For this review, take the finished solid that the model builds, in its own axes (mm). Face numbers are marked on the shaded views. A direction names the side the tool comes from. Round coordinates to 2 decimals unless told otherwise and drop trailing zeros. Loops run counter-clockwise (first coordinate to the right, second up) from the corner with the lowest first, then second, coordinate; pieces in that order, holes last.
1) Tool access review of the marked faces 1, 2 and 3: name each direction out of +Z, -Z, +X, -X, +Y, -Y from which nothing blocks a thin tool from reaching the whole face with its end or side.
2) Take a section at A-A (y = 15.5). State the section outline as (x, z) points, then the cut area to 3 significant figures.
3) Take a section at D-D (y = 35). State the section outline as (x, z) points, then the cut area to 3 significant figures.
4) Take a section at B-B (x = 62). State the section outline as (y, z) points, then the cut area to 3 significant figures.
5) Wall thickness on L1, parallel to X at y = 29.5, z = 12.5; L2, parallel to Y at x = -72, z = -15; L3, parallel to X at y = 12, z = 18: over which ranges is each line inside the solid? List them lowest first.
6) Mouldability with a two-part tool opening along X and no side actions: class the marked faces 4, 5 and 6 as pulls with the +X half, pulls with the -X half, needs draft (parallel to the pull), parting line crosses it, or undercut.
7) Insertion check: pin 1 (7 mm diameter, centred on y = 27, z = 1, fed in from +X); pin 2 (2 mm diameter, centred on y = 62, z = 10, fed in from +X); pin 3 (4 mm diameter, centred on x = -6.5, z = -5, fed in from +Y); pin 4 (8 mm diameter, centred on x = 14, y = 69.5, fed in from -Z). Each pin has a flat end and moves straight along its axis. Give the tip position at first contact, or say it passes through.
8) Take a section at C-C (z = -9). State the section outline as (x, y) points, then the cut area to 3 significant figures.
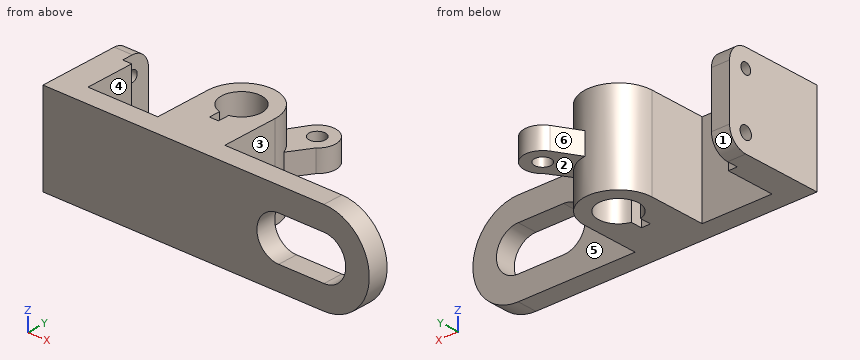
```python
from build123d import *

# Parameters (mm, degrees)
BASE_PLATE_11MM_DEPTH    = 11
UPRIGHT_BLOCK_DEPTH      = 50
CHANNEL_CUT_DEPTH        = 50
FRONT_WALL_12MM_DEPTH    = 6
WALL_HOLE_SKETCH_R       = 4.5
WALL_THROUGH_HOLE_DEPTH  = 69
BORE_KEYWAY_CUT_DEPTH    = 69
HOUSING_PAD_SKETCH_W     = 15
HOUSING_PAD_SKETCH_H     = 50
HOUSING_PAD_DEPTH        = 27
BORE_HOUSING_SKETCH_W    = 10
BORE_HOUSING_SKETCH_H    = 16
BORE_HOUSING_DEPTH       = 50
HOUSING_FILLET_R10_A_R   = 10
HOUSING_FILLET_R10_B_R   = 10
CROSS_HOLE_SKETCH_R      = 3.5
CROSS_HOLE_SKETCH_R_2    = 3
HOUSING_CROSS_HOLE_DEPTH = 40


with BuildPart() as part:
    # Base Plate Sketch → Base Plate 11mm (new body)
    with BuildSketch(Plane(origin=(0, 0, 0), x_dir=(1, 0, 0), z_dir=(0, 1, 0))):
        with BuildLine():
            Line((-77.5, 25), (-77.5, -25))
            Line((-77.5, -25), (77.5, -25))
            ThreePointArc((77.5, -25), (102.5, 0), (77.5, 25))
            Line((77.5, 25), (-77.5, 25))
        make_face()
    extrude(amount=BASE_PLATE_11MM_DEPTH)

    # Upright Block Sketch → Upright Block (add)
    with BuildSketch(Plane.XY.offset(25)):
        with BuildLine():
            ThreePointArc((13, 42), (-5.5, 60.5), (-24, 42))
            Line((-24, 42), (-24, 11))
            Line((-24, 11), (13, 11))
            Line((13, 11), (13, 42))
        make_face()
    extrude(amount=-UPRIGHT_BLOCK_DEPTH)

    # Channel Cut Sketch → Channel Cut (cut)
    with BuildSketch(Plane.XY.offset(25)):
        with BuildLine():
            Line((-5.5, 25), (-8, 25))
            Line((-8, 25), (-8, 31.287857357))
            ThreePointArc((-8, 31.287857357), (-5.5, 53), (-3, 31.287857357))
            Line((-3, 31.287857357), (-3, 25))
            Line((-3, 25), (-5.5, 25))
        make_face()
    extrude(amount=-CHANNEL_CUT_DEPTH, mode=Mode.SUBTRACT)

    # Front Wall Sketch → Front Wall 12mm (add, symmetric)
    with BuildSketch(Plane.XY):
        with BuildLine():
            Line((4.241132249, 73.293301112), (-3.376902326, 60.37777071))
            Line((-3.376902326, 60.37777071), (11.674130016, 48.877445616))
            Line((11.674130016, 48.877445616), (19.069800109, 60.379004757))
            ThreePointArc((19.069800109, 60.379004757), (19.421965671, 75.753931979), (4.241132249, 73.293301112))
        make_face()
    extrude(amount=FRONT_WALL_12MM_DEPTH, both=True)

    # Wall Hole Sketch → Wall Through Hole (cut)
    with BuildSketch(Plane.XY.offset(6)):
        with Locations((12.854445963, 68.212865417)):
            Circle(WALL_HOLE_SKETCH_R)
    extrude(amount=-WALL_THROUGH_HOLE_DEPTH, mode=Mode.SUBTRACT)

    # Bore Keyway Sketch → Bore Keyway Cut (cut)
    with BuildSketch(Plane(origin=(0, 11, 0), x_dir=(1, 0, 0), z_dir=(0, 1, 0))):
        with BuildLine():
            Line((52.5, 12), (77.5, 12))
            ThreePointArc((77.5, 12), (89.5, 0), (77.5, -12))
            Line((77.5, -12), (52.5, -12))
            ThreePointArc((52.5, -12), (40.5, 0), (52.5, 12))
        make_face()
    extrude(amount=-BORE_KEYWAY_CUT_DEPTH, mode=Mode.SUBTRACT)

    # Housing Pad Sketch → Housing Pad (add)
    with BuildSketch(Plane(origin=(0, 11, 0), x_dir=(1, 0, 0), z_dir=(0, 1, 0))):
        with Locations((-70, 0)):
            Rectangle(HOUSING_PAD_SKETCH_W, HOUSING_PAD_SKETCH_H)
    extrude(amount=HOUSING_PAD_DEPTH)

    # Bore Housing Sketch → Bore Housing (add)
    with BuildSketch(Plane.XY.offset(25)):
        with Locations((-72.5, 46)):
            Rectangle(BORE_HOUSING_SKETCH_W, BORE_HOUSING_SKETCH_H)
    extrude(amount=-BORE_HOUSING_DEPTH)

    # Housing Fillet R10 A
    housing_fillet_r10_a_edges = [part.edges().sort_by_distance(p)[0] for p in [
        (-72.5, 54, 25),
    ]]
    fillet(housing_fillet_r10_a_edges, radius=HOUSING_FILLET_R10_A_R)

    # Housing Fillet R10 B
    housing_fillet_r10_b_edges = [part.edges().sort_by_distance(p)[0] for p in [
        (-72.5, 54, -25),
    ]]
    fillet(housing_fillet_r10_b_edges, radius=HOUSING_FILLET_R10_B_R)

    # Cross Hole Sketch → Housing Cross Hole (cut)
    with BuildSketch(Plane.ZY.offset(77.5)):
        with Locations((-15, 44)):
            Circle(CROSS_HOLE_SKETCH_R)
        with Locations((15, 44)):
            Circle(CROSS_HOLE_SKETCH_R_2)
    extrude(amount=-HOUSING_CROSS_HOLE_DEPTH, mode=Mode.SUBTRACT)


solid = part.part
```
Response:
1. face 1: -Z, -X, +Y
1. face 2: -Z, +X, +Y
1. face 3: +Z, -Z, +X
2. outline: (-77.5, -25) - (-62.5, -25) - (-62.5, 25) - (-77.5, 25) - close; (-24, -25) - (13, -25) - (13, 25) - (-24, 25) - close
2. area: 2,600 mm2
3. outline: (-77.5, -25) - (-62.5, -25) - (-62.5, 25) - (-77.5, 25) - close; (-24, -25) - (-13.99, -25) - (-13.99, 25) - (-24, 25) - close; (2.99, -25) - (13, -25) - (13, 25) - (2.99, 25) - close
3. area: 1,750 mm2
4. outline: (0, -25) - (11, -25) - (11, -12) - (0, -12) - close; (0, 12) - (11, 12) - (11, 25) - (0, 25) - close
4. area: 286 mm2
5. L1: x = -77.5 to -62.5, -24 to -8, -3 to 13
5. L2: y = 0 to 40.5, 47.5 to 54
5. L3: x = -77.5 to -62.5, -24 to 13
6. face 4: undercut
6. face 5: needs draft
6. face 6: pulls with the -X half
7. pin 1: stops at x = 13
7. pin 2: passes through
7. pin 3: stops at y = 60.5
7. pin 4: stops at z = -6
8. outline: (-77.5, 0) - (44.56, 0) - (44.56, 11) - (13, 11) - (13, 42) arc R18.5 ccw to (-24, 42) - (-24, 11) - (-62.5, 11) - (-62.5, 38) - (-67.5, 38) - (-67.5, 54) - (-77.5, 54) - close; (85.44, 0) - (100.82, 0) - (100.82, 11) - (85.44, 11) - close; hole (-8, 25) - (-3, 25) - (-3, 31.29) arc R11 ccw (long way) to (-8, 31.29) - close
8. area: 3,350 mm2
